Read the model definition and answer for the solid it produces. Units are mm, in the model's axes. Face numbers are marked on the shaded views. Coordinates: 2 decimals unless noted, no trailing zeros. Order: outer loops, then holes, each group sorted by start corner. A loop starts at its lowest first (then second) coordinate and runs counter-clockwise, first axis right, second up. Notation, with made-up numbers: (89.5, -31) -> (97.5, -31) arc R26 ccw to (97.5, -10) -> close; hole circle Ø11 at (33.5, 5.25). An arc over 180 degrees is marked (long way). Answer in a Markdown table with one row per item.
from build123d import *

# Parameters (mm, degrees)
SKETCH_1_W          = 30
SKETCH_1_H          = 8
EXTRUDE_1_DEPTH     = 8
SKETCH_2_R          = 2.15
CUT_EXTRUDE_1_DEPTH = 21.498011819
CUT_EXTRUDE_2_DEPTH = 20.588803717


with BuildPart() as part:
    # 草图1 → 凸台-拉伸1 (new body)
    with BuildSketch(Plane.XY):
        with Locations((2.092936803, -1.249070632)):
            Rectangle(SKETCH_1_W, SKETCH_1_H)
    extrude(amount=EXTRUDE_1_DEPTH)

    # 草图2 → 切除-拉伸1 (cut, through all)
    with BuildSketch(Plane(origin=(0, 2.750929368, 0), x_dir=(1, 0, 0), z_dir=(0, 1, 0))):
        with Locations(Location((-7.907063197, -4, 0), (0, 0, 270))):
            Circle(SKETCH_2_R)
        with Locations(Location((12.092936803, -4, 0), (0, 0, 270))):
            Circle(SKETCH_2_R)
    extrude(amount=-CUT_EXTRUDE_1_DEPTH, mode=Mode.SUBTRACT)

    # 草图3 → 切除-拉伸2 (cut, through all)
    with BuildSketch(Plane.XY.offset(8)):
        with BuildLine():
            Line((2.746526641, 2.750929368), (3.439346964, 2.750929368))
            ThreePointArc((3.439346964, 2.750929368), (3.092936803, 2.550929368), (2.746526641, 2.750929368))
        make_face()
    extrude(amount=-CUT_EXTRUDE_2_DEPTH, mode=Mode.SUBTRACT)


solid = part.part
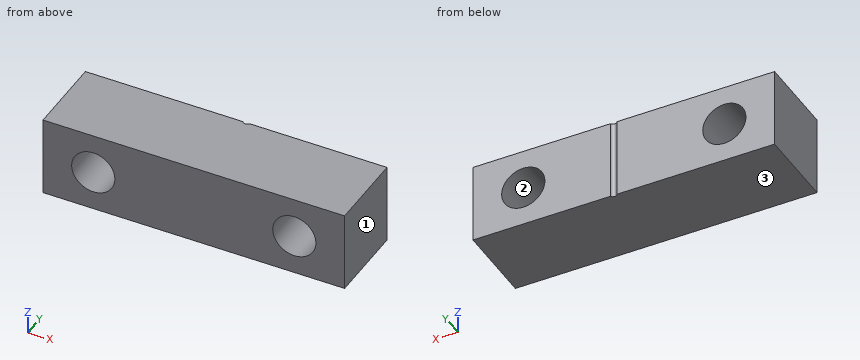
Q1. Consider line 1 (X direction, y = -2, z = 4); line 2 (X direction, y = -3.25, z = 2.5); line 3 (Z direction, x = 12.5, y = -2.75). Determine where each line is inside the solid, lowest interval first.
Outcome:
| item | result |
|---|---|
| line 1 | -12.91 to -10.06, -5.76 to 9.94, 14.24 to 17.09 |
| line 2 | -12.91 to -9.45, -6.37 to 10.55, 13.63 to 17.09 |
| line 3 | 0 to 1.89, 6.11 to 8 |
Q2. For a pull along X with two mould halves and no side action, classify the marked faces 1, 2 and 3 as pulls with the +X half, pulls with the -X half, needs draft (parallel to the pull), parting line crosses it, or undercut.
Outcome:
| item | result |
|---|---|
| face 1 | pulls with the +X half |
| face 2 | undercut |
| face 3 | needs draft |
Q3. The part is cut by section C-C (y = 2.25). Write down the section's boundary in (x, z), then the cut area to 3 significant figures.
Outcome:
| item | result |
|---|---|
| outline | (-12.91, 0) -> (17.09, 0) -> (17.09, 8) -> (-12.91, 8) -> close; hole circle Ø4.3 at (-7.91, 4); hole circle Ø4.3 at (12.09, 4) |
| area | 211 mm² |
Q4. The part is cut by section A-A (z = 4). Write down the section's boundary in (x, y), then the cut area to 3 significant figures.
Outcome:
| item | result |
|---|---|
| outline | (-12.91, -5.25) -> (-10.06, -5.25) -> (-10.06, 2.75) -> (-12.91, 2.75) -> close; (-5.76, -5.25) -> (9.94, -5.25) -> (9.94, 2.75) -> (3.44, 2.75) arc R0.4 cw to (2.75, 2.75) -> (-5.76, 2.75) -> close; (14.24, -5.25) -> (17.09, -5.25) -> (17.09, 2.75) -> (14.24, 2.75) -> close |
| area | 171 mm² |
Q5. The part is cut by section B-B (x = 11.75). Write down the section's boundary in (y, z).
Outcome:
| item | result |
|---|---|
| outline | (-5.25, 0) -> (2.75, 0) -> (2.75, 1.88) -> (-5.25, 1.88) -> close; (-5.25, 6.12) -> (2.75, 6.12) -> (2.75, 8) -> (-5.25, 8) -> close |
Q6. Given pin 1 (4 mm diameter, centred on x = 12.09, z = 4, fed in from +Y), flat-ended and moving along its own axis, determine where the tip first touches the part or whether it passes through.
Outcome:
| item | result |
|---|---|
| pin 1 | through |
